Geometry: see drawing. Coordinates: mm, zero at the bounding-box minimum. A direction names the side the tool comes from. Coordinates: 2 decimals unless noted, no trailing zeros. Loops run counter-clockwise (first coordinate to the right, second up) from the corner with the lowest first, then second, coordinate; pieces in that order, holes last. Notation, with made-up numbers: (84.25, -20.5) -> (88.25, -20.5) arc R19 ccw to (88.25, 13.5) -> close; hole circle Ø6 at (-14, 54.25). An arc over 180 degrees is marked (long way). One line per item, written item: value. Start each with the question number.
Item 1: Section query D-D on x = 1.85. Return loops of the section in (y, z), then the cut area to 3 significant figures.
Item 2: Section query A-A on y = 13.25. Return loops of the section in (x, z).
Item 3: Contact query for flat-ended pins moving along their axis: pin 1 Ø2 at (x, z) = (1.5, 21.5) entering from -Y; pin 2 Ø1 at (x, z) = (1, 3.5) entering from -Y; pin 3 Ø1.5 at (x, y) = (5.5, 23) entering from +Z. Output: stop coordinate, or through.
Item 4: Set-up query: the marked faces 1 and 2. Return all of +Z, -Z, +X, -X, +Y, -Y with unobstructed straight access to the full face (end or side cutting, diameter ignored); none if empty.
Item 5: Section query C-C on x = 5.5. Return loops of the section in (y, z), then the cut area to 3 significant figures.
Item 6: Mould query, pull axis Z, two halves, no side actions, for the marked faces 3, 4, 5 and 6. Classes: +Z half, -Z half, draft (parallel to the pull), parting line (faces both ways), or undercut.
Item 7: Ray query, probe 1 along Y at (x, z) = (5.2, 13.25); probe 2 along Y at (x, z) = (3.15, 13.25); probe 3 along Y at (x, z) = (0.35, 9.5). Return the intervals inside material, ascending. Write a range as from..to.
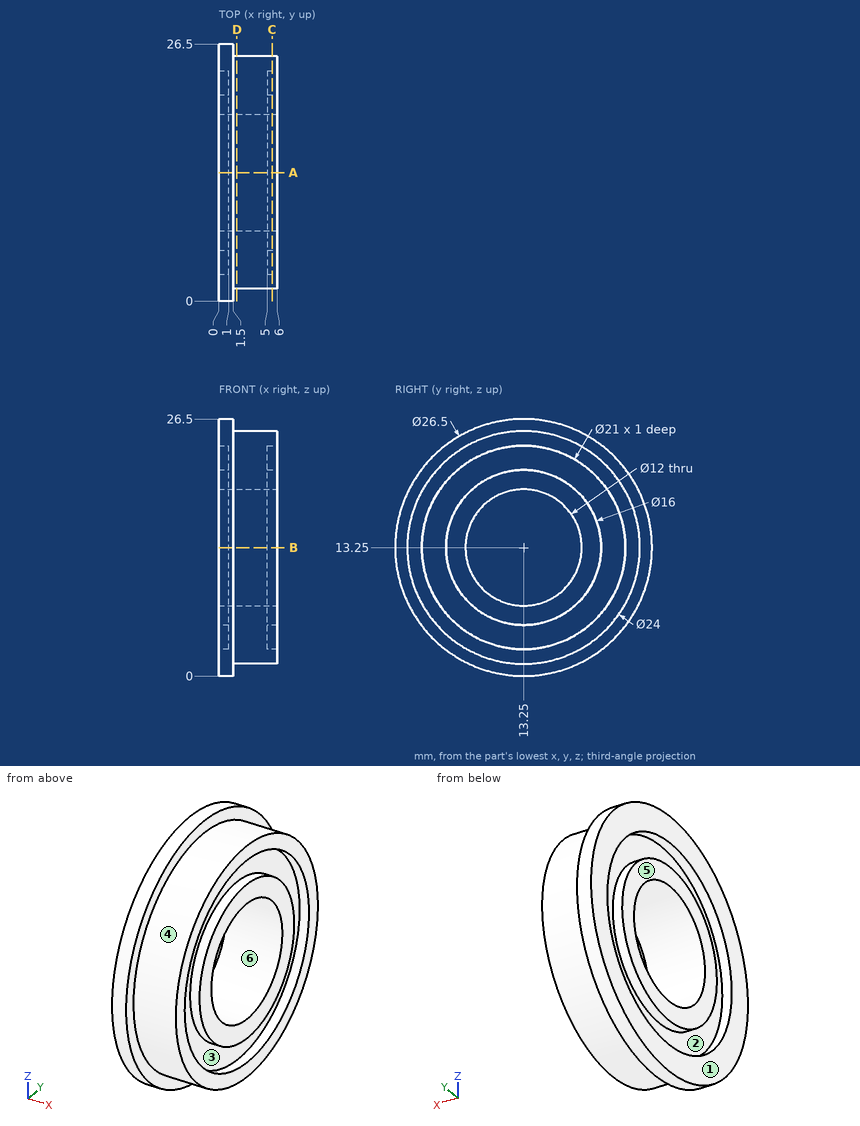
Reply:
1. outline: circle Ø24 at (13.25, 13.25); hole circle Ø12 at (13.25, 13.25)
1. area: 339 mm²
2. outline: (0, 0) -> (1.5, 0) -> (1.5, 1.25) -> (6, 1.25) -> (6, 2.75) -> (5, 2.75) -> (5, 5.25) -> (6, 5.25) -> (6, 7.25) -> (0, 7.25) -> (0, 5.25) -> (1, 5.25) -> (1, 2.75) -> (0, 2.75) -> close; (0, 19.25) -> (6, 19.25) -> (6, 21.25) -> (5, 21.25) -> (5, 23.75) -> (6, 23.75) -> (6, 25.25) -> (1.5, 25.25) -> (1.5, 26.5) -> (0, 26.5) -> (0, 23.75) -> (1, 23.75) -> (1, 21.25) -> (0, 21.25) -> close
3. pin 1: stops at y = 2.16
3. pin 2: stops at y = 3.76
3. pin 3: stops at z = 21.19
4. face 1: +Z, -Z, -X, +Y, -Y
4. face 2: -X
5. outline: circle Ø24 at (13.25, 13.25); circle Ø16 at (13.25, 13.25); hole circle Ø21 at (13.25, 13.25); hole circle Ø12 at (13.25, 13.25)
5. area: 194 mm²
6. face 3: undercut
6. face 4: parting line
6. face 5: draft
6. face 6: undercut
7. probe 1: y = 1.25..2.75, 5.25..7.25, 19.25..21.25, 23.75..25.25
7. probe 2: y = 1.25..7.25, 19.25..25.25
7. probe 3: y = 0.54..3.44, 6.18..8.57, 17.93..20.32, 23.06..25.96
